Here's how the part is built. I have some questions about the finished solid (model axes, mm). A direction names the side the tool comes from. Round coordinates to 2 decimals unless told otherwise and drop trailing zeros. Loops run counter-clockwise (first coordinate to the right, second up) from the corner with the lowest first, then second, coordinate; pieces in that order, holes last. Notation, with made-up numbers: M 83.5,-27 L 104.5,-27 A26 cw 104.5,-9 Z; hole C 74,27 d6. An arc over 180 degrees is marked long. Answer as a JSON object with one key per item and string values.
from build123d import *

# Parameters (mm, degrees)
SKETCH1_W                                        = 240
SKETCH1_H                                        = 65
BOSS_EXTRUDE1_DEPTH                              = 12
CUT_EXTRUDE1_DEPTH                               = 125.900960765
CUT_EXTRUDE1_DEPTH_BACK                          = 125.900960765
SKETCH2_W                                        = 95
SKETCH2_H                                        = 18
FILLET1_R                                        = 5
HOLE_FOR_SOCKET_HEAD_CAP_SCREW_TYPE1_D           = 6.6
HOLE_FOR_SOCKET_HEAD_CAP_SCREW_TYPE1_CBORE_D     = 11
HOLE_FOR_SOCKET_HEAD_CAP_SCREW_TYPE1_CBORE_DEPTH = 6.8
F_4_5_4_5_DIAMETER_HOLE1_D                       = 4.5
CHAMFER1_SIZE                                    = 2


with BuildPart() as part:
    # Sketch1 → Boss-Extrude1 (new body)
    with BuildSketch(Plane.XY):
        Rectangle(SKETCH1_W, SKETCH1_H)
    extrude(amount=BOSS_EXTRUDE1_DEPTH)

    # Sketch2 → Cut-Extrude1 (cut, two sides: drawn at the far end of the back side and taken through both)
    with BuildSketch(Plane.XY.offset(12).offset(-CUT_EXTRUDE1_DEPTH_BACK)):
        with Locations((-72.5, 23.5)):
            Rectangle(SKETCH2_W, SKETCH2_H)
        with Locations((72.5, 23.5)):
            Rectangle(SKETCH2_W, SKETCH2_H)
        with Locations((72.5, -23.5)):
            Rectangle(SKETCH2_W, SKETCH2_H)
        with Locations((-72.5, -23.5)):
            Rectangle(SKETCH2_W, SKETCH2_H)
    extrude(amount=CUT_EXTRUDE1_DEPTH + CUT_EXTRUDE1_DEPTH_BACK, mode=Mode.SUBTRACT)

    # Fillet1
    fillet1_edges = [part.edges().sort_by_distance(p)[0] for p in [
        (-25, -32.5, 6),
        (-25, -14.5, 6),
        (25, -32.5, 6),
        (25, -14.5, 6),
        (25, 32.5, 6),
        (25, 14.5, 6),
        (-25, 32.5, 6),
        (-25, 14.5, 6),
    ]]
    fillet(fillet1_edges, radius=FILLET1_R)

    # Hole for socket head cap screw, type1 (through all)
    with Locations(Plane(origin=(0, 0, 0), x_dir=(-1, 0, 0), z_dir=(0, 0, -1))):
        with Locations((15.202795796, -15.202795796), (0, -21.5), (-15.202795796, -15.202795796), (-21.5, 0), (-15.202795796, 15.202795796), (0, 21.5), (15.202795796, 15.202795796), (21.5, 0)):
            CounterBoreHole(HOLE_FOR_SOCKET_HEAD_CAP_SCREW_TYPE1_D / 2, HOLE_FOR_SOCKET_HEAD_CAP_SCREW_TYPE1_CBORE_D / 2, HOLE_FOR_SOCKET_HEAD_CAP_SCREW_TYPE1_CBORE_DEPTH)

    # Ø4.5 (4.5) Diameter Hole1 (through all)
    with Locations(Plane.XY.offset(12)):
        with Locations((-93, -8.5), (-108, -8.5), (-93, 8.5), (-108, 8.5)):
            f_4_5_4_5_diameter_hole1 = Hole(F_4_5_4_5_DIAMETER_HOLE1_D / 2)

    # Mirror1: Ø4.5 (4.5) Diameter Hole1 across plane
    add(f_4_5_4_5_diameter_hole1.mirror(Plane(origin=(0, 0, 0), x_dir=(0, 0, 1), z_dir=(1, 0, 0))), mode=Mode.SUBTRACT)

    # Chamfer1
    chamfer1_edges = [part.edges().sort_by_distance(p)[0] for p in [
        (-120, -14.5, 6),
        (120, -14.5, 6),
        (120, 14.5, 6),
        (-120, 14.5, 6),
    ]]
    chamfer(chamfer1_edges, length=CHAMFER1_SIZE)


solid = part.part
Item 1: I want a section at D-D, the plane x = -62.5. Please give me the cut outline in (y, z), then the cut area to 3 significant figures.
Resolved:
{"outline": "M -14.5,0 L 14.5,0 L 14.5,12 L -14.5,12 Z", "area": "348 mm²"}
Item 2: I want a section at A-A, the plane y = 0. Please give me the cut outline in (x, z).
Resolved:
{"outline": "M -120,0 L -27,0 L -27,6.8 L -24.8,6.8 L -24.8,12 L -120,12 Z; M -18.2,6.8 L -16,6.8 L -16,0 L 16,0 L 16,6.8 L 18.2,6.8 L 18.2,12 L -18.2,12 Z; M 24.8,6.8 L 27,6.8 L 27,0 L 120,0 L 120,12 L 24.8,12 Z"}
Item 3: I'm going to push flat-ended pins straight in: pin 1 Ø2.5 at (y, z) = (21.5, 7) entering from +X; pin 2 Ø10 at (x, y) = (15.2, 15.2) entering from -Z; pin 3 Ø6 at (y, z) = (-18, 1.5) entering from -X. Where does each tip first touch, or does it pass through?
Resolved:
{"pin 1": "x = 25", "pin 2": "z = 6.8", "pin 3": "x = -27.82"}
Item 4: On a 3-axis mill with a long thin cutter (end or side, diameter ignored), from which of +Z, -Z, +X, -X, +Y, -Y can I reach the whole of each face in a straight line? I mean faces 1 (the face through (4.05, -17.78, 3.35)), 2 (the face through (-75, 14.5, 6)), 3 (the face through (-75, -14.5, 6)), 4 (the face through (73, 14.5, 6)), 5 (the face through (73, -14.5, 6)). Say none if no direction works.
Resolved:
{"face 1": "-Z", "face 2": "+Z, -Z, -X, +Y", "face 3": "+Z, -Z, -X, -Y", "face 4": "+Z, -Z, +X, +Y", "face 5": "+Z, -Z, +X, -Y"}
Item 5: I want a section at C-C, the plane x = -108. Please give me the cut outline in (y, z).
Resolved:
{"outline": "M -14.5,0 L -10.75,0 L -10.75,12 L -14.5,12 Z; M -6.25,0 L 6.25,0 L 6.25,12 L -6.25,12 Z; M 10.75,0 L 14.5,0 L 14.5,12 L 10.75,12 Z"}
Item 6: I want a section at B-B, the plane x = 0. Please give me the cut outline in (y, z), then the cut area to 3 significant figures.
Resolved:
{"outline": "M -32.5,0 L -27,0 L -27,6.8 L -24.8,6.8 L -24.8,12 L -32.5,12 Z; M -18.2,6.8 L -16,6.8 L -16,0 L 16,0 L 16,6.8 L 18.2,6.8 L 18.2,12 L -18.2,12 Z; M 24.8,6.8 L 27,6.8 L 27,0 L 32.5,0 L 32.5,12 L 24.8,12 Z", "area": "562 mm²"}
Item 7: Please list where these lines run through material, in increasing order: probe 1 along Y at (x, z) = (0, 8.7); probe 2 along Y at (x, z) = (-1.5, 9.75); probe 3 along Y at (x, z) = (102, 7.5). Write a range as from..to.
Resolved:
{"probe 1": "-32.5..-24.8, -18.2..18.2, 24.8..32.5", "probe 2": "-32.5..-24.44, -18.56..18.56, 24.44..32.5", "probe 3": "-14.5..14.5"}
